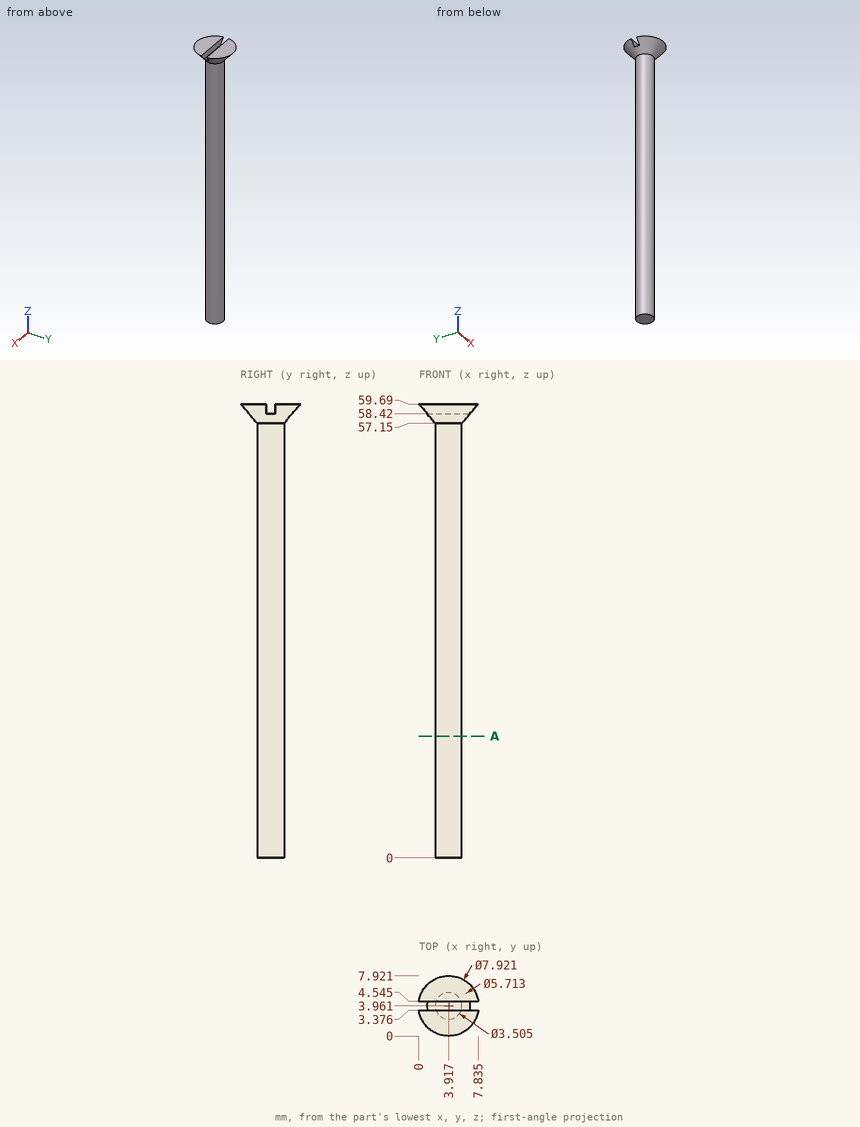
Check sheet for the drawn part. Datum: minimum x, y, z corner. Units: mm. Give positions to 0.01 mm unless a question says otherwise; leave off trailing zeros. Order: outer loops, then holes, each group sorted by start corner. A loop starts at its lowest first (then second) coordinate and runs counter-clockwise, first axis right, second up. Notation, with made-up numbers: (-22.5, 36.5) -> (12.5, 36.5) arc R29 ccw to (12.5, 61.5) -> close; hole circle Ø7 at (-15, 37). An arc over 180 degrees is marked (long way). Return JSON: item names as keys, results as strings.
1. Go/stop test with flat-tipped pins: P1, Ø4, axis at x = 5, z = 35.5, coming from the +Y side; P2, Ø0.6, axis at x = 5, z = 59, coming from the +Y side; P3, Ø1, axis at x = 6, z = 59, coming from the -Y side (1 decimal). Record where each tip stops, or that it passes through.
From the geometry:
{"P1": "y = 5.71", "P2": "y = 7.43", "P3": "y = 0.7"}
2. Material ranges on probe 1 along X at (y, z) = (4, 19.5) (1 decimal); probe 2 along Z at (x, y) = (5.5, 3.75); probe 3 along Z at (x, y) = (6.25, 2), recorded low to high. Write a range as [from, to].
From the geometry:
{"probe 1": "[2.2, 5.7]", "probe 2": "[0, 58.42]", "probe 3": "[58.64, 59.69]"}
3. Cross-section at A-A, the plane z = 16. Record the cut outline in (x, y) (1 decimal).
From the geometry:
{"outline": "circle Ø3.5 at (3.9, 4)"}
